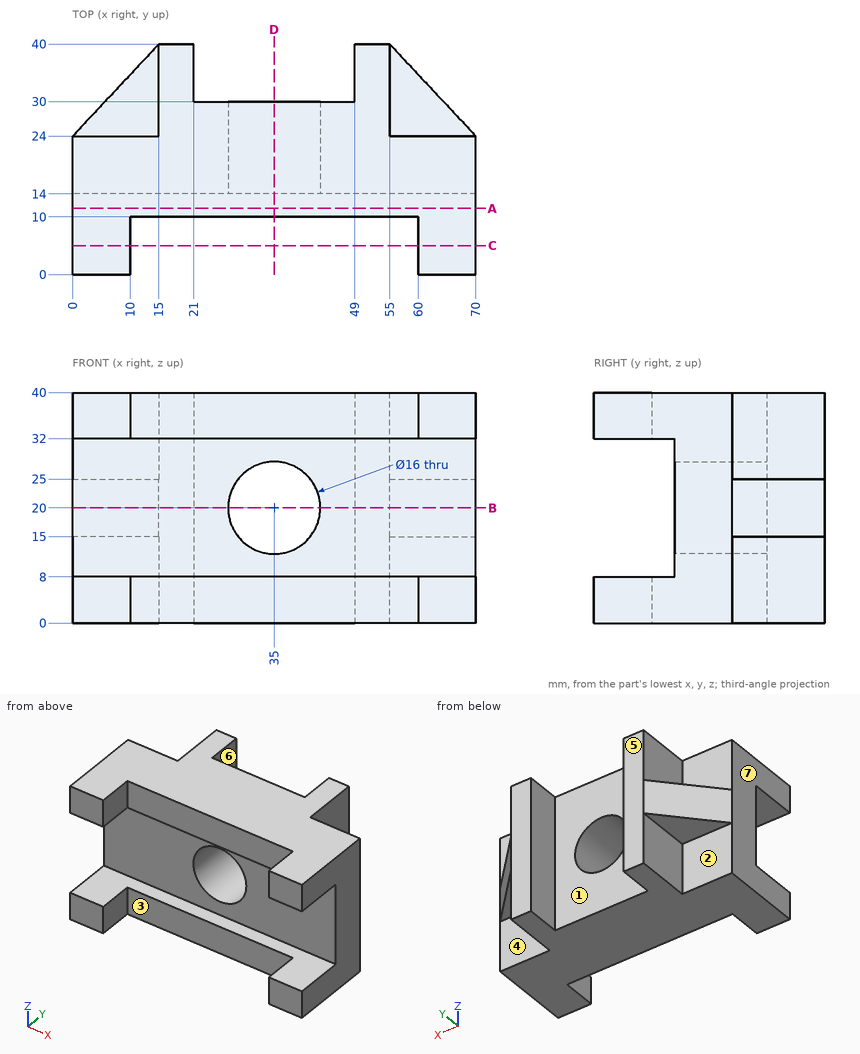
For this review, use the dimensioned drawing (mm, ordinates from the lowest corner) and the shaded views. A direction names the side the tool comes from. Round coordinates to 2 decimals unless told otherwise and drop trailing zeros. Write each loop counter-clockwise with the first axis right and the second up, starting at its lowest first coordinate (ties: lowest second). Pieces come first, ordered by that corner, then holes. Notation, with made-up numbers: (49.25, 30) - (90.25, 30) arc R22 cw to (90.25, 49) - close; hole circle Ø1 at (-26.75, 45.5). An arc over 180 degrees is marked (long way). One line per item, written item: value. Start each with the question number.
1. Consider section A-A on y = 11.5. Write out the cut boundary in (x, z), and give its area (3 significant figures).
2. Consider section B-B on z = 20. Write out the cut boundary in (x, y), and give its area (3 significant figures).
3. Machinability: for the marked faces 1, 2, 3 and 4, which of the approach directions +Z, -Z, +X, -X, +Y, -Y give a long, thin tool a straight path to every point of the face, cutting with its end or side? Answer none if there is none.
4. Clearance check with flat-ended pins moving along their axes: P1, Ø3, axis at y = 34, z = 28.5, coming from the +X side; P2, Ø10, axis at y = 32.5, z = 31.5, coming from the -X side; P3, Ø7, axis at x = 21.5, y = 7, coming from the -Z side; P4, Ø4, axis at x = 40.5, z = 37, coming from the -Y side. State where each tip first meets the part, or that it passes through.
5. Consider section C-C on y = 5. Write out the cut boundary in (x, z).
6. The part is to be moulded in two halves that separate along X. For the marked faces 5, 6 and 7, say which applies: released by +X, released by -X, zero draft, split by the parting line, or undercut.
7. To check wall thickness, follow L1, parallel to Z at x = 9.5, y = 9.5; L2, parallel to Z at x = 35, y = 24; L3, parallel to Y at x = 66, z = 12. State the ranges of each line that lie inside material, in increasing order. Write a range as from..to.
8. Consider section D-D on x = 35. Write out the cut boundary in (y, z), and give its area (3 significant figures).
Checks:
1. outline: (0, 0) - (70, 0) - (70, 8) - (0, 8) - close; (0, 32) - (70, 32) - (70, 40) - (0, 40) - close
1. area: 1,120 mm^2
2. outline: (0, 14) - (27, 14) - (27, 30) - (21, 30) - (21, 40) - (15, 40) - (0, 24) - close; (43, 14) - (70, 14) - (70, 24) - (55, 40) - (49, 40) - (49, 30) - (43, 30) - close
2. area: 1,040 mm^2
3. face 1: +Z, -Z, +Y
3. face 2: -Z, -X, +Y
3. face 3: +Z, -Z, -Y
3. face 4: -Z, +X, +Y
4. P1: stops at x = 55
4. P2: stops at x = 15
4. P3: stops at z = 0
4. P4: stops at y = 10
5. outline: (0, 0) - (10, 0) - (10, 8) - (0, 8) - close; (0, 32) - (10, 32) - (10, 40) - (0, 40) - close; (60, 0) - (70, 0) - (70, 8) - (60, 8) - close; (60, 32) - (70, 32) - (70, 40) - (60, 40) - close
6. face 5: zero draft
6. face 6: undercut
6. face 7: released by -X
7. L1: z = 0..8, 32..40
7. L2: z = 0..12, 28..40
7. L3: y = 14..24
8. outline: (10, 0) - (30, 0) - (30, 12) - (14, 12) - (14, 8) - (10, 8) - close; (10, 32) - (14, 32) - (14, 28) - (30, 28) - (30, 40) - (10, 40) - close
8. area: 448 mm^2
